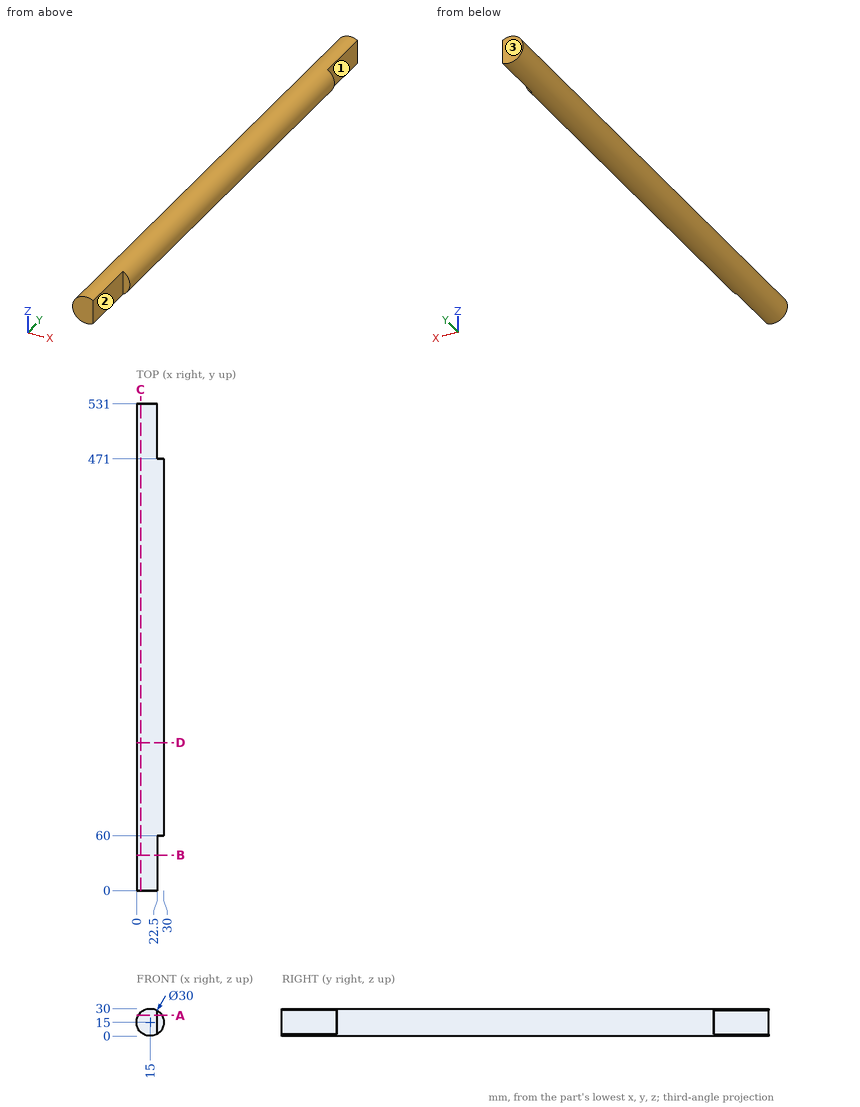
Verification items for this drawing (mm, ordinates from the low corner). A direction names the side the tool comes from. Give positions to 0.01 mm unless a question says otherwise; leave off trailing zeros. Write each loop counter-clockwise with the first axis right and the second up, starting at its lowest first coordinate (ties: lowest second). Pieces come first, ordered by that corner, then holes.
1) Section check C-C, the plane x = 4.5. Record the boundary of the cut face in (y, z).
2) Section check A-A, the plane z = 22.5. Record the boundary of the cut face in (x, y), and give its area (3 significant figures).
3) Material ranges on L1, parallel to X at y = 425, z = 15.5; L2, parallel to Z at x = 14.75, y = 222; L3, parallel to Y at x = 23.5, z = 4, recorded low to high.
4) Section check B-B, the plane y = 38.5. Record the boundary of the cut face in (x, z), and give its area (3 significant figures).
5) Access from +Z, -Z, +X, -X, +Y, -Y to the whole of each face (thin tool, end or side, straight path). Record for the marked faces 1, 2 and 3.
6) Section check D-D, the plane y = 161.5. Record the boundary of the cut face in (x, z), and give its area (3 significant figures).
7) Gauge pin test, flat ends, axial feed: pin 1 (1 mm diameter, centred on y = 272, z = 9.5, fed in from +X); pin 2 (6 mm diameter, centred on x = 26, z = 14, fed in from -Y); pin 3 (2 mm diameter, centred on x = 26, z = 16, fed in from +Y). Record the tip position at first contact, or that the pin passes through.
Computed:
1. outline: (0, 4.29) - (531, 4.29) - (531, 25.71) - (0, 25.71) - close
2. outline: (2.01, 0) - (22.5, 0) - (22.5, 60) - (27.99, 60) - (27.99, 471) - (22.5, 471) - (22.5, 531) - (2.01, 531) - close
2. area: 13,100 mm2
3. L1: x = 0.01 to 29.99
3. L2: z = 0 to 30
3. L3: y = 60 to 471
4. outline: (22.5, 2.01) - (22.5, 27.99) arc R15 ccw (long way) to start
4. area: 569 mm2
5. face 1: +Z, -Z, +X, +Y
5. face 2: +Z, -Z, +X, -Y
5. face 3: +Z, -Z, +X, -X, +Y
6. outline: circle Ø30 at (15, 15)
6. area: 707 mm2
7. pin 1: stops at x = 29.14
7. pin 2: stops at y = 60
7. pin 3: stops at y = 471
